The listing builds one solid part. Answer for the finished solid, in the listing's coordinates (mm). A direction names the side the tool comes from. Coordinates: 2 decimals unless noted, no trailing zeros. Loops run counter-clockwise (first coordinate to the right, second up) from the corner with the lowest first, then second, coordinate; pieces in that order, holes last. Notation, with made-up numbers: (-28.75, 79.5) - (30.25, 79.5) arc R11 cw to (30.25, 86.5) - close; hole circle Ø11 at (50.25, 88). An arc over 180 degrees is marked (long way). Use one line per item in the form item = value. Start each with the question number.
```python
from build123d import *

# Parameters (mm, degrees)
SKETCH_1_W      = 30
SKETCH_1_H      = 60
EXTRUDE_1_DEPTH = 415
SHELL_1_T       = -2


with BuildPart() as part:
    # 草图1 → 凸台-拉伸1 (new, symmetric)
    with BuildSketch(Plane.XY):
        Rectangle(SKETCH_1_W, SKETCH_1_H)
    extrude(amount=EXTRUDE_1_DEPTH, both=True)

    # 抽壳1
    shell_1_openings = [part.faces().sort_by_distance(p)[0] for p in [
        (0, 0, 415),
        (0, 0, -415),
        (0, 30, 0),
    ]]
    offset(amount=SHELL_1_T, openings=shell_1_openings, kind=Kind.INTERSECTION)


solid = part.part
```
(1) Find the intervals of material crossed by probe 1 along X at (y, z) = (-6, -194); probe 2 along Y at (x, z) = (-6.5, 144), in increasing order. Write a range as from..to.
(2) For faces 1 (the face through (-13, 1, 6)), 2 (the face through (0, -30, 6)), determine the directions among +Z, -Z, +X, -X, +Y, -Y from which every point of the face is accessible in a straight line to the end or side of a thin tool.
(3) Determine the mould class of faces 3 (the face through (0, -28, 6)), 4 (the face through (-13.4, -6.5, -415)), 5 (the face through (-15, 0, 6)) for opening direction X: +X half, -X half, draft (parallel to the pull), parting line (faces both ways), or undercut.
(4) A cutting plane is placed at B-B (z = -310.5). Determine the outline of the cut face in (x, y).
(5) A cutting plane is placed at C-C (x = 5.25). Determine the outline of the cut face in (y, z), then the cut area to 3 significant figures.
(6) A cutting plane is placed at A-A (y = -6.5). Determine the outline of the cut face in (x, z).
(7) This flat-tipped pin is pushed along its axis until it touches: pin 1 Ø8 at (x, y) = (8.5, 6.5) entering from +Z. Where does it stop, or does it pass through?
Evaluation:
q1.probe_1 = -15..-13, 13..15
q1.probe_2 = -30..-28
q2.face_1 = +Z, -Z, +Y
q2.face_2 = +Z, -Z, +X, -X, -Y
q3.face_3 = undercut
q3.face_4 = draft
q3.face_5 = -X half
q4.outline = (-15, -30) - (15, -30) - (15, 30) - (13, 30) - (13, -28) - (-13, -28) - (-13, 30) - (-15, 30) - close
q5.outline = (-30, -415) - (-28, -415) - (-28, 415) - (-30, 415) - close
q5.area = 1,660 mm^2
q6.outline = (-15, -415) - (-13, -415) - (-13, 415) - (-15, 415) - close; (13, -415) - (15, -415) - (15, 415) - (13, 415) - close
q7.pin_1 = through
